from build123d import *

# Parameters (mm, degrees)
SKETCH1_W                  = 130
SKETCH1_H                  = 116
BOSS_EXTRUDE1_DEPTH        = 1
SKETCH2_R                  = 9
CUT_EXTRUDE1_DEPTH         = 88.120606058
LPATTERN1_COUNT            = 3
LPATTERN1_PITCH            = 38
LPATTERN1_COUNT_DIR2       = 5
LPATTERN1_PITCH_DIR2       = 22.5
CHAMFER1_SIZE              = 2
F_3_5_3_5_DIAMETER_HOLE1_D = 3.5
LPATTERN2_COUNT            = 4
LPATTERN2_PITCH            = 40
LPATTERN2_COUNT_DIR2       = 4
LPATTERN2_PITCH_DIR2       = 35


with BuildPart() as part:
    # Sketch1 → Boss-Extrude1 (new body)
    with BuildSketch(Plane(origin=(0, 0, 0), x_dir=(1, 0, 0), z_dir=(0, 1, 0))):
        Rectangle(SKETCH1_W, SKETCH1_H)
    extrude(amount=BOSS_EXTRUDE1_DEPTH)

    # Sketch2 → Cut-Extrude1 (cut, through all)
    with BuildSketch(Plane(origin=(0, 1, 0), x_dir=(1, 0, 0), z_dir=(0, 1, 0))):
        with Locations(Location((45, -38, 0), (0, 0, 270))):
            Circle(SKETCH2_R)
    cut_extrude1 = extrude(amount=-CUT_EXTRUDE1_DEPTH, mode=Mode.SUBTRACT)

    # LPattern1: Cut-Extrude1 3 × 5, 7 skipped
    with Locations(*[(-j * LPATTERN1_PITCH_DIR2, 0, -i * LPATTERN1_PITCH) for i in range(LPATTERN1_COUNT) for j in range(LPATTERN1_COUNT_DIR2) if (i, j) not in ((0, 0), (0, 1), (0, 3), (1, 0), (1, 2), (1, 4), (2, 1), (2, 3))]):
        add(cut_extrude1, mode=Mode.SUBTRACT)

    # Chamfer1
    chamfer1_edges = [part.edges().sort_by_distance(p)[0] for p in [
        (65, 0.5, 58),
        (-65, 0.5, 58),
        (-65, 0.5, -58),
        (65, 0.5, -58),
    ]]
    chamfer(chamfer1_edges, length=CHAMFER1_SIZE)

    # Ø3.5 (3.5) Diameter Hole1 (through all)
    with Locations(Plane(origin=(0, 1, 0), x_dir=(1, 0, 0), z_dir=(0, 1, 0))):
        with Locations((60, -52.5)):
            f_3_5_3_5_diameter_hole1 = Hole(F_3_5_3_5_DIAMETER_HOLE1_D / 2)

    # LPattern2: 3.5 _3.5_ Diameter Hole1 4 × 4
    with Locations(*[(-i * LPATTERN2_PITCH, 0, -j * LPATTERN2_PITCH_DIR2) for i in range(LPATTERN2_COUNT) for j in range(LPATTERN2_COUNT_DIR2) if (i, j) != (0, 0)]):
        add(f_3_5_3_5_diameter_hole1, mode=Mode.SUBTRACT)


solid = part.part
Can you work these out from the model? Positions are in its coordinate system, mm. Give positions to 0.01 mm unless a question says otherwise; leave off trailing zeros. Loops run counter-clockwise (first coordinate to the right, second up) from the corner with the lowest first, then second, coordinate; pieces in that order, holes last. Notation, with made-up numbers: (74.25, -39) -> (87.25, -39) arc R23 ccw to (87.25, -29) -> close; hole circle Ø6 at (29, 36.25). An arc over 180 degrees is marked (long way). Use one line per item in the form item = value.
1) If we section it at D-D (z = -38): Please give me the cut outline in (x, y).
Answers:
outline = (-65, 0) -> (-54, 0) -> (-54, 1) -> (-65, 1) -> close; (-36, 0) -> (-9, 0) -> (-9, 1) -> (-36, 1) -> close; (9, 0) -> (36, 0) -> (36, 1) -> (9, 1) -> close; (54, 0) -> (65, 0) -> (65, 1) -> (54, 1) -> close
2) We'd pull the mould along Z, two halves only. Please class faces 1 (the face through (-1, 0, -1)), 2 (the face through (-61.617, 0.493, -51.83)), 3 (the face through (-38.917, 0.507, -44.633)): released by +Z, released by -Z, zero draft, split by the parting line, or undercut.
Answers:
face_1 = zero draft
face_2 = undercut
face_3 = undercut
3) Will this pin go through, and if not, where does the flat tip stop? pin 1 (3 mm diameter, centred on x = 60, z = 52.5, fed in from +Y).
Answers:
pin_1 = through
4) If we section it at B-B (y = 0.4): Count the separate pieces of the cut face and the enclosed holes in it, plus the area to 3 significant figures.
Answers:
separate_pieces = 1
enclosed_holes = 24
area = 12,900 mm²
5) If we section it at A-A (x = -45): Please give me the cut outline in (y, z), plus the area to 3 significant figures.
Answers:
outline = (0, -58) -> (1, -58) -> (1, -47) -> (0, -47) -> close; (0, -29) -> (1, -29) -> (1, 29) -> (0, 29) -> close; (0, 47) -> (1, 47) -> (1, 58) -> (0, 58) -> close
area = 80.0 mm²
6) I need wall thicknesses on line 1 along Z through (x, y) = (60, 0.55); line 2 along X through (y, z) = (0.4, 0); line 3 along Z through (x, y) = (0.5, 0.8). Which ranges of each line are inside material? Lowest first, please.
Answers:
line_1 = -58 to -54.25, -50.75 to -19.25, -15.75 to 15.75, 19.25 to 50.75, 54.25 to 58
line_2 = -65 to -31.5, -13.5 to 13.5, 31.5 to 65
line_3 = -58 to -46.99, -29.01 to 29.01, 46.99 to 58
7) If we section it at C-C (z = 52.5): Please give me the cut outline in (x, y).
Answers:
outline = (-65, 0) -> (-61.75, 0) -> (-61.75, 1) -> (-65, 1) -> close; (-58.25, 0) -> (-21.75, 0) -> (-21.75, 1) -> (-58.25, 1) -> close; (-18.25, 0) -> (18.25, 0) -> (18.25, 1) -> (-18.25, 1) -> close; (21.75, 0) -> (58.25, 0) -> (58.25, 1) -> (21.75, 1) -> close; (61.75, 0) -> (65, 0) -> (65, 1) -> (61.75, 1) -> close
